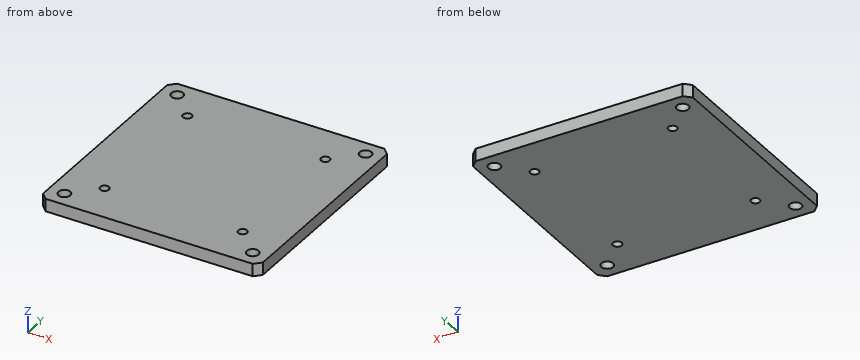
from build123d import *

# Parameters (mm, degrees)
SKETCH_1_W                  = 350
SKETCH_1_H                  = 350
EXTRUDE_1_DEPTH             = 20
HOLE_WIZARD_M16_1_D         = 14
HOLE_WIZARD_M16_1_DEPTH     = 42
HOLE_WIZARD_M16_1_TIP       = 4.206024333
HOLE_WIZARD_19_0_19_1_D     = 19
HOLE_WIZARD_19_0_19_1_DEPTH = 25
HOLE_WIZARD_19_0_19_1_TIP   = 5.708175881
CHAMFER_1_SIZE              = 10


with BuildPart() as part:
    # 草图1 → 凸台-拉伸1 (new body)
    with BuildSketch(Plane.XY):
        Rectangle(SKETCH_1_W, SKETCH_1_H)
    extrude(amount=EXTRUDE_1_DEPTH)

    # M16 螺纹孔1
    with Locations(Plane.XY.offset(20)):
        with Locations((110, 110), (-110, -110), (-110, 110), (110, -110)):
            Hole(HOLE_WIZARD_M16_1_D / 2, depth=HOLE_WIZARD_M16_1_DEPTH)
            with Locations((0, 0, -(HOLE_WIZARD_M16_1_DEPTH + HOLE_WIZARD_M16_1_TIP / 2))):  # 118° drill point
                Cone(0, HOLE_WIZARD_M16_1_D / 2, HOLE_WIZARD_M16_1_TIP, mode=Mode.SUBTRACT)

    # Ø19.0 (19) 直径孔1
    with Locations(Plane.XY.offset(20)):
        with Locations((150, 150), (-150, -150), (-150, 150), (150, -150)):
            Hole(HOLE_WIZARD_19_0_19_1_D / 2, depth=HOLE_WIZARD_19_0_19_1_DEPTH)
            with Locations((0, 0, -(HOLE_WIZARD_19_0_19_1_DEPTH + HOLE_WIZARD_19_0_19_1_TIP / 2))):  # 118° drill point
                Cone(0, HOLE_WIZARD_19_0_19_1_D / 2, HOLE_WIZARD_19_0_19_1_TIP, mode=Mode.SUBTRACT)

    # 倒角1
    chamfer_1_edges = [part.edges().sort_by_distance(p)[0] for p in [
        (175, -175, 10),
        (-175, -175, 10),
        (-175, 175, 10),
        (175, 175, 10),
    ]]
    chamfer(chamfer_1_edges, length=CHAMFER_1_SIZE)


solid = part.part
For this review, take the finished solid that the model builds, in its own axes (mm). Give positions to 0.01 mm unless a question says otherwise; leave off trailing zeros. Order: outer loops, then holes, each group sorted by start corner. A loop starts at its lowest first (then second) coordinate and runs counter-clockwise, first axis right, second up. Notation, with made-up numbers: M 34.5,77.5 L 45.5,77.5 A20 ccw 45.5,95.5 Z; hole C 71,18 d9. An arc over 180 degrees is marked long. Answer in a Markdown table with one row per item. Add a question column.
(1) Consider section A-A on z = 9.75. Give the number of separate pieces and of enclosed holes in the cut face, and give its area (3 significant figures).
(2) Wall thickness on probe 1 along Y at (x, z) = (110, 8); probe 2 along X at (y, z) = (109.5, 14); probe 3 along Y at (x, z) = (-149, 5.75): over which ranges is each line inside the solid? List them lowest first. Write a range as [from, to].
(3) Consider section B-B on y = -150. State the section outline as (x, z) points, and give its area (3 significant figures).
(4) Consider section C-C on x = 110. State the section outline as (y, z) points, and give its area (3 significant figures).
(5) For pin 1 (11 mm diameter, centred on x = -110, y = -110, fed in from +Z), flat-tipped, find the tip position at first contact; note if it passes through.
Evaluation:
| question | item | result |
|---|---|---|
| 1 | separate pieces | 1 |
| 1 | enclosed holes | 8 |
| 1 | area | 121,000 mm^2 |
| 2 | probe 1 | y = [-175, -117], [-103, 103], [117, 175] |
| 2 | probe 2 | x = [-175, -116.98], [-103.02, 103.02], [116.98, 175] |
| 2 | probe 3 | y = [-175, -159.45], [-140.55, 140.55], [159.45, 175] |
| 3 | outline | M -175,0 L -159.5,0 L -159.5,20 L -175,20 Z; M -140.5,0 L 140.5,0 L 140.5,20 L -140.5,20 Z; M 159.5,0 L 175,0 L 175,20 L 159.5,20 Z |
| 3 | area | 6,240 mm^2 |
| 4 | outline | M -175,0 L -117,0 L -117,20 L -175,20 Z; M -103,0 L 103,0 L 103,20 L -103,20 Z; M 117,0 L 175,0 L 175,20 L 117,20 Z |
| 4 | area | 6,440 mm^2 |
| 5 | pin 1 | passes through |
